Source: CAD feature listing. Evaluate the final solid. Frame: model axes, mm. A direction names the side the tool comes from. Give positions to 0.01 mm unless a question says otherwise; leave off trailing zeros. Write each loop counter-clockwise with the first axis right and the second up, starting at its lowest first coordinate (ties: lowest second). Pieces come first, ordered by that corner, then holes. Notation, with made-up numbers: (86.5, 87) - (100.5, 87) arc R17 cw to (100.5, 92) - close; hole circle Ø5 at (-6, 74). An arc over 180 degrees is marked (long way). One line per question, with ' | ' between items. Start each with the question number.
(1) Draft query along Z for faces 6 (the flat face through (0, -7, 28)), 7 (the flat face through (0, -4.25, 21)), 8 (the flat face through (0, 4.25, 21)), 9 (the flat face through (-0.1, 10.2, 0)). Return one class per face: +Z half, -Z half, draft (parallel to the pull), parting line (faces both ways), or undercut.
(2) Section A-A, the plane x = -6.5. Return loops of the section in (y, z).
(3) Section C-C, the plane x = 1.25. Return loops of the section in (y, z).
(4) Pin query (flat end, axial travel): pin 1 (6 mm diameter, centred on x = 4.5, z = 28.5, fed in from -Y); pin 2 (14.5 mm diameter, centred on x = 0.5, z = 27.5, fed in from +Y); pin 3 (3 mm diameter, centred on y = 4, z = 24.5, fed in from -X). Return the tip coordinate at first contact, or that it passes through.
(5) Access query for faces 1 (the cylindrical face through (2.17, -9.76, 7.4)), 2 (the flat face through (0, -5, 20)), 3 (the flat face through (4.25, 0, 21)), 4 (the flat face through (-4.25, 0, 21)), 5 (the flat face through (0, 7, 28)). Directions: +Z, -Z, +X, -X, +Y, -Y. A direction counts if a zero-diameter tool reaches every point of the face in a straight line with its end or side. Return the directions, or none.
(6) Ray query, line 1 (Z direction, x = -5.5, y = 1.25); line 2 (Y direction, x = 0, z = 7.5); line 3 (Z direction, x = 9, y = 8.5). Return the intervals inside material, ascending. Write a range as [from, to].
(7) Section D-D, the plane z = 7. Return loops of the section in (x, y).
(8) Section B-B, the plane y = 0. Return loops of the section in (x, z).
```python
from build123d import *

# Parameters (mm, degrees)
SKETCH_1_R          = 12.5
EXTRUDE_1_DEPTH     = 20
SKETCH_2_W          = 8.5
SKETCH_2_H          = 8.5
EXTRUDE_2_DEPTH     = 1.7
SKETCH_3_W          = 14
SKETCH_3_H          = 14
EXTRUDE_3_DEPTH     = 13.17
SKETCH_4_R          = 10
CUT_EXTRUDE_1_DEPTH = 15
CHAMFER_1_SIZE      = 0.5


with BuildPart() as part:
    # 草图1 → 凸台-拉伸1 (new body)
    with BuildSketch(Plane.XY):
        Circle(SKETCH_1_R)
    extrude(amount=EXTRUDE_1_DEPTH)

    # 草图2 → 凸台-拉伸2 (add)
    with BuildSketch(Plane.XY.offset(20)):
        Rectangle(SKETCH_2_W, SKETCH_2_H)
    extrude(amount=EXTRUDE_2_DEPTH)

    # 草图3 → 凸台-拉伸3 (add)
    with BuildSketch(Plane.XY.offset(21.7)):
        Rectangle(SKETCH_3_W, SKETCH_3_H)
    extrude(amount=EXTRUDE_3_DEPTH)

    # 草图4 → 切除-拉伸1 (cut)
    with BuildSketch(Plane(origin=(0, 0, 0), x_dir=(-1, 0, 0), z_dir=(0, 0, -1))):
        Circle(SKETCH_4_R)
    extrude(amount=-CUT_EXTRUDE_1_DEPTH, mode=Mode.SUBTRACT)

    # 倒角1
    chamfer_1_edges = [part.edges().sort_by_distance(p)[0] for p in [
        (4.25, 0, 20),
        (0, 4.25, 20),
        (-4.25, 0, 20),
        (0, -4.25, 20),
    ]]
    chamfer(chamfer_1_edges, length=CHAMFER_1_SIZE)


solid = part.part
```
Check sheet entries:
1) face 6: draft | face 7: undercut | face 8: undercut | face 9: -Z half
2) outline: (-10.68, 0) - (-7.6, 0) - (-7.6, 15) - (7.6, 15) - (7.6, 0) - (10.68, 0) - (10.68, 20) - (-10.68, 20) - close; (-7, 21.7) - (7, 21.7) - (7, 34.87) - (-7, 34.87) - close
3) outline: (-12.44, 0) - (-9.92, 0) - (-9.92, 15) - (9.92, 15) - (9.92, 0) - (12.44, 0) - (12.44, 20) - (4.75, 20) - (4.25, 20.5) - (4.25, 21.7) - (7, 21.7) - (7, 34.87) - (-7, 34.87) - (-7, 21.7) - (-4.25, 21.7) - (-4.25, 20.5) - (-4.75, 20) - (-12.44, 20) - close
4) pin 1: y = -7 | pin 2: y = 7 | pin 3: x = -7
5) face 1: -Z | face 2: none | face 3: +X, +Y, -Y | face 4: -X, +Y, -Y | face 5: +Z, +X, -X, +Y
6) line 1: [15, 20], [21.7, 34.87] | line 2: [-12.5, -10], [10, 12.5] | line 3: [0, 20]
7) outline: circle Ø25 at (0, 0); hole circle Ø20 at (0, 0)
8) outline: (-12.5, 0) - (-10, 0) - (-10, 15) - (10, 15) - (10, 0) - (12.5, 0) - (12.5, 20) - (4.75, 20) - (4.25, 20.5) - (4.25, 21.7) - (7, 21.7) - (7, 34.87) - (-7, 34.87) - (-7, 21.7) - (-4.25, 21.7) - (-4.25, 20.5) - (-4.75, 20) - (-12.5, 20) - close
